Check sheet for the modelled part. Datum: model origin and axes. Units: mm. A direction names the side the tool comes from. Round coordinates to 2 decimals unless told otherwise and drop trailing zeros. Write each loop counter-clockwise with the first axis right and the second up, starting at its lowest first coordinate (ties: lowest second). Pieces come first, ordered by that corner, then holes. Notation, with made-up numbers: (-31.75, 37) -> (-11.75, 37) arc R23 ccw to (-11.75, 48) -> close; hole circle Ø2 at (-5.75, -7). An arc over 180 degrees is marked (long way). Use one line per item in the form item = value. Start each with the question number.
```python
from build123d import *

# Parameters (mm, degrees)
EXTRUDE_1_REACH = 69.614
SKETCH_2_W      = 0.974227423
SKETCH_2_H      = 0.5


with BuildPart() as part:
    # 草图1 → 旋转1 (revolve)
    with BuildSketch(Plane.XY, mode=Mode.PRIVATE) as revolve_1_sk:
        with BuildLine():
            Line((-4.6, 0), (-4, 0))
            Line((-4, 0), (-4, 1))
            Line((-4, 1), (-3.5, 1))
            Line((-3.5, 1), (-3.5, 2.5))
            Line((-3.5, 2.5), (-4, 2.5))
            Line((-4, 2.5), (-4, 4.3))
            Line((-4, 4.3), (-3.5, 4.3))
            Line((-3.5, 4.3), (-3.5, 5.8))
            Line((-3.5, 5.8), (-4, 5.8))
            Line((-4, 5.8), (-4, 7.3))
            Line((-4, 7.3), (-3.5, 7.3))
            Line((-3.5, 7.3), (-3.5, 9.1))
            Line((-3.5, 9.1), (-4, 9.1))
            Line((-4, 9.1), (-4, 10))
            Line((-4, 10), (-2.75, 10))
            Line((-2.75, 10), (-2.575500592, 64.3))
            ThreePointArc((-2.575500592, 64.3), (-2.282607373, 65.007106781), (-1.575500592, 65.3))
            Line((-1.575500592, 65.3), (0, 65.3))
            Line((0, 65.3), (0, 67.3))
            Line((0, 67.3), (-0.391399138, 67.3))
            ThreePointArc((-0.391399138, 67.3), (-2.852382856, 66.288686228), (-3.891179873, 63.839176651))
            Line((-3.891179873, 63.839176651), (-3.969072705, 58.3))
            Line((-3.969072705, 58.3), (-3.25, 58.3))
            Line((-3.25, 58.3), (-3.25, 57.8))
            Line((-3.25, 57.8), (-3.974609916, 57.8))
            Line((-3.974609916, 57.8), (-3.985684336, 56.8))
            Line((-3.985684336, 56.8), (-3.25, 56.8))
            Line((-3.25, 56.8), (-3.25, 56.3))
            Line((-3.25, 56.3), (-3.985684336, 56.3))
            Line((-3.985684336, 56.3), (-4.6, 0))
        make_face()
    revolve(revolve_1_sk.sketch.rotate(Axis((0, 0, 0), (0, 1, 0)), 270), axis=Axis((0, 0, 0), (0, 1, 0)))

    # 凸台-拉伸1: up to this face of the body (flat: up to its plane)
    extrude_1_end = Plane(part.part.faces().sort_by_distance((0, 7.3, 3.886862915))[0])
    # 草图2 → 凸台-拉伸1 (add, up to the picked face)
    with BuildSketch(Plane.XZ, mode=Mode.PRIVATE) as extrude_1_sk1:
        with Locations((-3.887113712, 0)):
            Rectangle(SKETCH_2_W, SKETCH_2_H)
    extrude_1_tool1 = split(extrude(extrude_1_sk1.sketch, amount=-EXTRUDE_1_REACH, mode=Mode.PRIVATE), bisect_by=extrude_1_end, keep=Keep.BOTH, mode=Mode.PRIVATE)
    # 草图2 → 凸台-拉伸1 (add, up to the picked face)
    with BuildSketch(Plane.XZ, mode=Mode.PRIVATE) as extrude_1_sk2:
        with Locations((3.887113712, 0)):
            Rectangle(SKETCH_2_W, SKETCH_2_H)
    extrude_1_tool2 = split(extrude(extrude_1_sk2.sketch, amount=-EXTRUDE_1_REACH, mode=Mode.PRIVATE), bisect_by=extrude_1_end, keep=Keep.BOTH, mode=Mode.PRIVATE)
    add(extrude_1_tool1.solids().sort_by(Axis((-3.887114, 0, 0), (0, 1, 0)))[0])
    add(extrude_1_tool2.solids().sort_by(Axis((3.887114, 0, 0), (0, 1, 0)))[0])


solid = part.part
```
1. Depth check by flat-ended pin: pin 1 (1.5 mm diameter, centred on x = -1, z = 2.5, fed in from -Y); pin 2 (1.9 mm diameter, centred on x = 1.5, z = 2.5, fed in from -Y); pin 3 (0.6 mm diameter, centred on y = 2.5, z = 0, fed in from -X); pin 4 (4 mm diameter, centred on x = -1, z = 3, fed in from -Y). Enter the tip coordinate at first touch or a pass-through.
2. Scan lines: probe 1 along Y at (x, z) = (-0.5, 3.5); probe 2 along Y at (x, z) = (-2.5, 2.25); probe 3 along Y at (x, z) = (0.75, -3.25). Record each from-to range of solid material in increasing order.
3. Sectioned sample at A-A (y = 18). Enter the section's corners in (x, z).
4. Tool access check on faces 1 (the face through (3, 10, 1)), 2 (the face through (-0.8, 37.53, -2.54)). Record the directions out of +Z, -Z, +X, -X, +Y, -Y that give a thin tool (end or side, any length) a straight path to the whole face; none if there is none.
5. Sectioned sample at B-B (y = 33). Enter the section's corners in (x, z).
Returned:
q1.pin_1 = 10
q1.pin_2 = 1
q1.pin_3 = -4.58
q1.pin_4 = 0
q2.probe_1 = 1 to 2.5, 4.3 to 5.8, 7.3 to 9.1, 10 to 56.3, 56.8 to 57.8, 58.3 to 65.34
q2.probe_2 = 10 to 56.3, 56.8 to 57.8, 58.3 to 65.65
q2.probe_3 = 10 to 56.3, 56.8 to 57.8, 58.3 to 65.69
q3.outline = circle Ø8.81 at (0, 0); hole circle Ø5.45 at (0, 0)
q4.face_1 = none
q4.face_2 = -Y
q5.outline = circle Ø8.48 at (0, 0); hole circle Ø5.35 at (0, 0)
